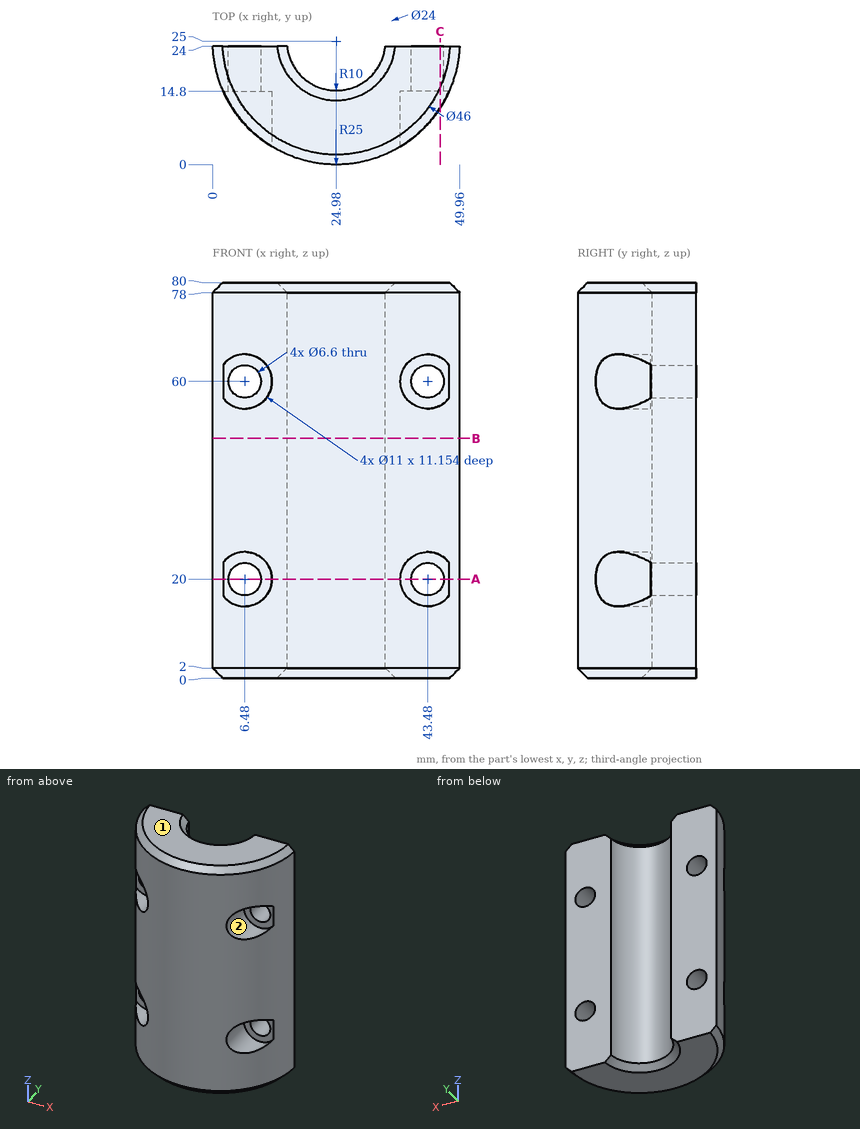
Can you work these out from the drawing? Everything is in mm from the part's minimum corner. A direction names the side the tool comes from. Round coordinates to 2 decimals unless told otherwise and drop trailing zeros. Loops run counter-clockwise (first coordinate to the right, second up) from the corner with the lowest first, then second, coordinate; pieces in that order, holes last. Notation, with made-up numbers: (-34, -19) - (23, -19) arc R25 cw to (23, 10) - close; hole circle Ø2 at (34, 7). An arc over 180 degrees is marked (long way). Write item = value, one per line. Start each with the question number.
(1) For P1, Ø3, axis at x = 40.5, z = 19.5, coming from the -Y side; P2, Ø4, axis at y = 12.5, z = 27.5, coming from the -X side; P3, Ø1, axis at y = 19.5, z = 33, coming from the -X side (3 decimals); P4, Ø5.5, axis at x = 43.48, z = 60, coming from the +Y side, each with a flat end and sliding along its axis, tell me the tip position at first contact or that it passes through.
(2) For the marked faces 1 and 2, which set-ups out of +Z, -Z, +X, -X, +Y, -Y let a thin tool reach every point of the face, with its end or its side?
(3) If I drill on probe 1 along X at (y, z) = (21.5, 60); probe 2 along X at (y, z) = (12.75, 20); probe 3 along X at (y, z) = (19.5, 20), over which ranges is the centre line in solid material (lowest first)? Write a range as [from, to].
(4) If we section it at A-A (z = 20): Please give me the cut outline in (x, y), and give its area (3 significant figures).
(5) If we section it at B-B (z = 48.5): Please give me the cut outline in (x, y), and give its area (3 significant figures).
(6) If we section it at C-C (x = 46): Give the number of separate pieces and of enclosed holes in the cut face, and give its area (3 significant figures).
Ans:
q1.P1 = 14.8
q1.P2 = 2.29
q1.P3 = 0.485
q1.P4 = through
q2.face_1 = +Z, +X, -X, +Y, -Y
q2.face_2 = -Y
q3.probe_1 = [0.23, 3.18], [9.78, 15.61], [34.35, 40.18], [46.78, 49.73]
q3.probe_2 = [11.98, 37.98]
q3.probe_3 = [0.59, 3.18], [9.78, 16.63], [33.33, 40.18], [46.78, 49.37]
q4.outline = (0, 24) arc R25 ccw to (2.16, 14.8) - (3.18, 14.8) - (3.18, 24) - close; (9.78, 14.8) - (11.98, 14.8) - (11.98, 3.65) arc R25 ccw to (37.98, 3.65) - (37.98, 14.8) - (40.18, 14.8) - (40.18, 24) - (34.93, 24) arc R10 cw to (15.03, 24) - (9.78, 24) - close; (46.78, 14.8) - (47.8, 14.8) arc R25 ccw to (49.96, 24) - (46.78, 24) - close
q4.area = 541 mm²
q5.outline = (0, 24) arc R25 ccw to (49.96, 24) - (34.93, 24) arc R10 cw to (15.03, 24) - close
q5.area = 795 mm²
q6.separate_pieces = 3
q6.enclosed_holes = 0
q6.area = 851 mm²
